Source: CAD feature listing. Evaluate the final solid. Frame: model axes, mm. Face numbers are marked on the shaded views. A direction names the side the tool comes from. Round coordinates to 2 decimals unless told otherwise and drop trailing zeros. Order: outer loops, then holes, each group sorted by start corner. A loop starts at its lowest first (then second) coordinate and runs counter-clockwise, first axis right, second up. Notation, with made-up numbers: (-12, -19) - (45, -19) arc R31 cw to (45, 9) - close; hole circle Ø3 at (21, 10.5). An arc over 180 degrees is marked (long way). Put each result on its own line as item: value. Start each with the question number.
1) Section B-B on y = 90. Output: boundary loops of the cut face in (x, z), then the cut area to 3 significant figures.
2) Section A-A on y = 153.5. Output: boundary loops of the cut face in (x, z), then the cut area to 3 significant figures.
3) Contact query for flat-ended pins moving along their axis: P1, Ø0.8, axis at x = -4, z = 4.5, coming from the -Y side; P2, Ø3, axis at x = 3, y = 87, coming from the +Z side; P3, Ø1.1, axis at x = 1.5, z = -5.5, coming from the +Y side; P4, Ø2, axis at x = -8.5, y = 69.5, coming from the +Z side. Output: stop coordinate, or through.
4) Access query for the marked faces 5, 6, 7 and 8. Directions: +Z, -Z, +X, -X, +Y, -Y. A direction counts if a zero-diameter tool reaches every point of the face in a straight line with its end or side. Return the directions, or none.
5) Mould query, pull axis Y, two halves, no side actions, for the marked faces 1, 2, 3 and 4. Classes: +Y half, -Y half, draft (parallel to the pull), parting line (faces both ways), or undercut.
6) Line query: probe 1 along Y at (x, z) = (-6.25, 7); probe 2 along Y at (x, z) = (3.5, 11); probe 3 along Y at (x, z) = (4.5, -6). Output: solid intervals per line, ascending. Write a range as [from, to].
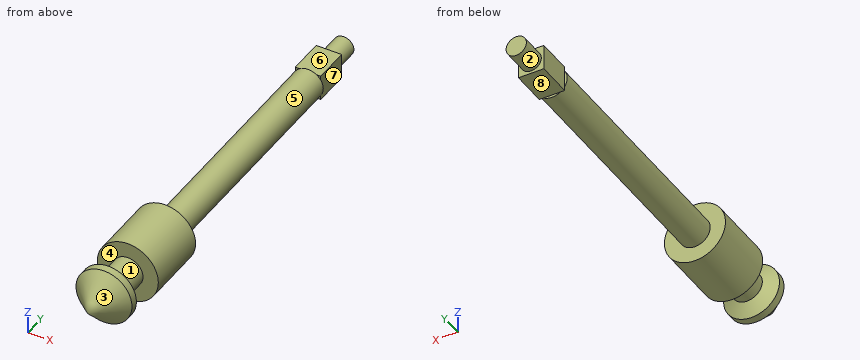
```python
from build123d import *

# Parameters (mm, degrees)
SKETCH2_W           = 10
SKETCH2_H           = 10
BOSS_EXTRUDE1_DEPTH = 14
SKETCH3_R           = 4
BOSS_EXTRUDE2_DEPTH = 10


with BuildPart() as part:
    # Sketch1 → Revolve1 (revolve)
    with BuildSketch(Plane.XY, mode=Mode.PRIVATE) as revolve1_sk:
        Polygon((0, 0), (-11, 11), (-11, 14), (-6, 17), (-6, 27), (-12, 27), (-12, 52), (-6, 52), (-6, 148), (0, 148), align=None)
    revolve(revolve1_sk.sketch.rotate(Axis((0, -1000, 0), (0, 1, 0)), 180), axis=Axis((0, -1000, 0), (0, 1, 0)))

    # Sketch2 → Boss-Extrude1 (add)
    with BuildSketch(Plane(origin=(0, 148, 0), x_dir=(1, 0, 0), z_dir=(0, 1, 0))):
        Rectangle(SKETCH2_W, SKETCH2_H)
    extrude(amount=BOSS_EXTRUDE1_DEPTH)

    # Sketch3 → Boss-Extrude2 (add)
    with BuildSketch(Plane(origin=(0, 162, 0), x_dir=(1, 0, 0), z_dir=(0, 1, 0))):
        Circle(SKETCH3_R)
    extrude(amount=BOSS_EXTRUDE2_DEPTH)


solid = part.part
```
Answer sheet:
1. outline: circle Ø12 at (0, 0)
1. area: 113 mm^2
2. outline: (-5, -5) - (5, -5) - (5, 5) - (-5, 5) - close
2. area: 100 mm^2
3. P1: y = 5.62
3. P2: z = 5.81
3. P3: y = 162
3. P4: through
4. face 5: none
4. face 6: +Z, +X, -X, +Y
4. face 7: +Z, -Z, +X, +Y
4. face 8: -Z, +X, -X, +Y
5. face 1: undercut
5. face 2: draft
5. face 3: -Y half
5. face 4: undercut
6. probe 1: [9.38, 14.97], [27, 52]
6. probe 2: [27, 52]
6. probe 3: [7.5, 16.1], [27, 52]
